Read the model definition and answer for the solid it produces. Units are mm, in the model's axes. A direction names the side the tool comes from. Coordinates: 2 decimals unless noted, no trailing zeros. Write each loop counter-clockwise with the first axis right and the second up, starting at its lowest first coordinate (ties: lowest second). Pieces come first, ordered by that corner, then holes. Notation, with made-up numbers: (-33.5, -6) - (-24.5, -6) arc R28 cw to (-24.5, 20) - close; hole circle Ø4 at (-35.5, 63.5). An arc over 180 degrees is marked (long way). Return JSON: item names as keys, results as strings.
```python
from build123d import *

# Parameters (mm, degrees)
BOSS_EXTRUDE1_DEPTH = 400
CUT_EXTRUDE1_REACH  = 426.264


with BuildPart() as part:
    # Sketch2 → Boss-Extrude1 (new, symmetric)
    with BuildSketch(Plane(origin=(0, 0, 0), x_dir=(1, 0, 0), z_dir=(0, 1, 0))):
        with BuildLine():
            Line((7.875, -1.525), (92.125, -1.525))
            ThreePointArc((92.125, -1.525), (97.693465902, 0.781534098), (100, 6.35))
            Line((100, 6.35), (100, 90.6))
            ThreePointArc((100, 90.6), (97.693465902, 96.168465902), (92.125, 98.475))
            Line((92.125, 98.475), (7.875, 98.475))
            ThreePointArc((7.875, 98.475), (2.306534098, 96.168465902), (0, 90.6))
            Line((0, 90.6), (0, 6.35))
            ThreePointArc((0, 6.35), (2.306534098, 0.781534098), (7.875, -1.525))
        make_face()
        with BuildLine():
            Line((12.6, 4.775), (87.4, 4.775))
            ThreePointArc((87.4, 4.775), (91.854772721, 6.620227279), (93.7, 11.075))
            Line((93.7, 11.075), (93.7, 85.875))
            ThreePointArc((93.7, 85.875), (91.854772721, 90.329772721), (87.4, 92.175))
            Line((87.4, 92.175), (12.6, 92.175))
            ThreePointArc((12.6, 92.175), (8.145227279, 90.329772721), (6.3, 85.875))
            Line((6.3, 85.875), (6.3, 11.075))
            ThreePointArc((6.3, 11.075), (8.145227279, 6.620227279), (12.6, 4.775))
        make_face(mode=Mode.SUBTRACT)
    extrude(amount=BOSS_EXTRUDE1_DEPTH, both=True)

    # Sketch4 → Cut-Extrude1 (cut, up to next)
    with BuildSketch(Plane.XY.offset(1.525), mode=Mode.PRIVATE) as cut_extrude1_sk1:
        Polygon((100, 400), (0, 376), (0, 400), align=None)
    cut_extrude1_tool1 = extrude(cut_extrude1_sk1.sketch, amount=-CUT_EXTRUDE1_REACH, mode=Mode.PRIVATE) & part.part
    add(cut_extrude1_tool1.solids().sort_by_distance((33.333333, 392, 1.525))[0], mode=Mode.SUBTRACT)


solid = part.part
```
(1) A cutting plane is placed at C-C (y = 274). Determine the outline of the cut face in (x, z) (3 decimals).
Answer:
{"outline": "(0, -90.6) arc R7.875 ccw to (7.875, -98.475) - (92.125, -98.475) arc R7.875 ccw to (100, -90.6) - (100, -6.35) arc R7.875 ccw to (92.125, 1.525) - (7.875, 1.525) arc R7.875 ccw to (0, -6.35) - close; hole (6.3, -85.875) arc R6.3 ccw to (12.6, -92.175) - (87.4, -92.175) arc R6.3 ccw to (93.7, -85.875) - (93.7, -11.075) arc R6.3 ccw to (87.4, -4.775) - (12.6, -4.775) arc R6.3 ccw to (6.3, -11.075) - close"}
(2) Determine the mould class of faces 3 (the face through (51, 5, -98.475)), 4 (the face through (50.7, 388.17, -3.33)), 5 (the face through (49, 4, -4.775)) for opening direction X: +X half, -X half, draft (parallel to the pull), parting line (faces both ways), or undercut.
Answer:
{"face 3": "draft", "face 4": "-X half", "face 5": "undercut"}
(3) Straight lines are drawn through the part: line 1 (Z direction, x = 62, y = -317.5) (3 decimals); line 2 (X direction, y = 180, z = -62); line 3 (X direction, y = -25.5, z = -87). For each, find the intervals that lie inside material, in ascending order. Write a range as from..to.
Answer:
{"line 1": "-98.475..-92.175, -4.775..1.525", "line 2": "0..6.3, 93.7..100", "line 3": "0..6.4, 93.6..100"}
(4) A cutting plane is placed at A-A (x = 59.5). Determine the outline of the cut face in (y, z) (3 decimals), and give its area (3 significant figures).
Answer:
{"outline": "(-400, -98.475) - (390.28, -98.475) - (390.28, -92.175) - (-400, -92.175) - close; (-400, -4.775) - (390.28, -4.775) - (390.28, 1.525) - (-400, 1.525) - close", "area": "9,960 mm²"}
(5) A cutting plane is placed at B-B (z = -19). Determine the outline of the cut face in (x, y), and give its area (3 significant figures).
Answer:
{"outline": "(0, -400) - (6.3, -400) - (6.3, 377.51) - (0, 376) - close; (93.7, -400) - (100, -400) - (100, 400) - (93.7, 398.49) - close", "area": "9,930 mm²"}
(6) Which of the six approach directions +Z, -Z, +X, -X, +Y, -Y give full straight-line access (tool end or side, diameter ignored) to faces 1 (the face through (51, 4, -92.175)), 2 (the face through (49, 5, 1.525))?
Answer:
{"face 1": "+Y, -Y", "face 2": "+Z, +X, -X, +Y, -Y"}
